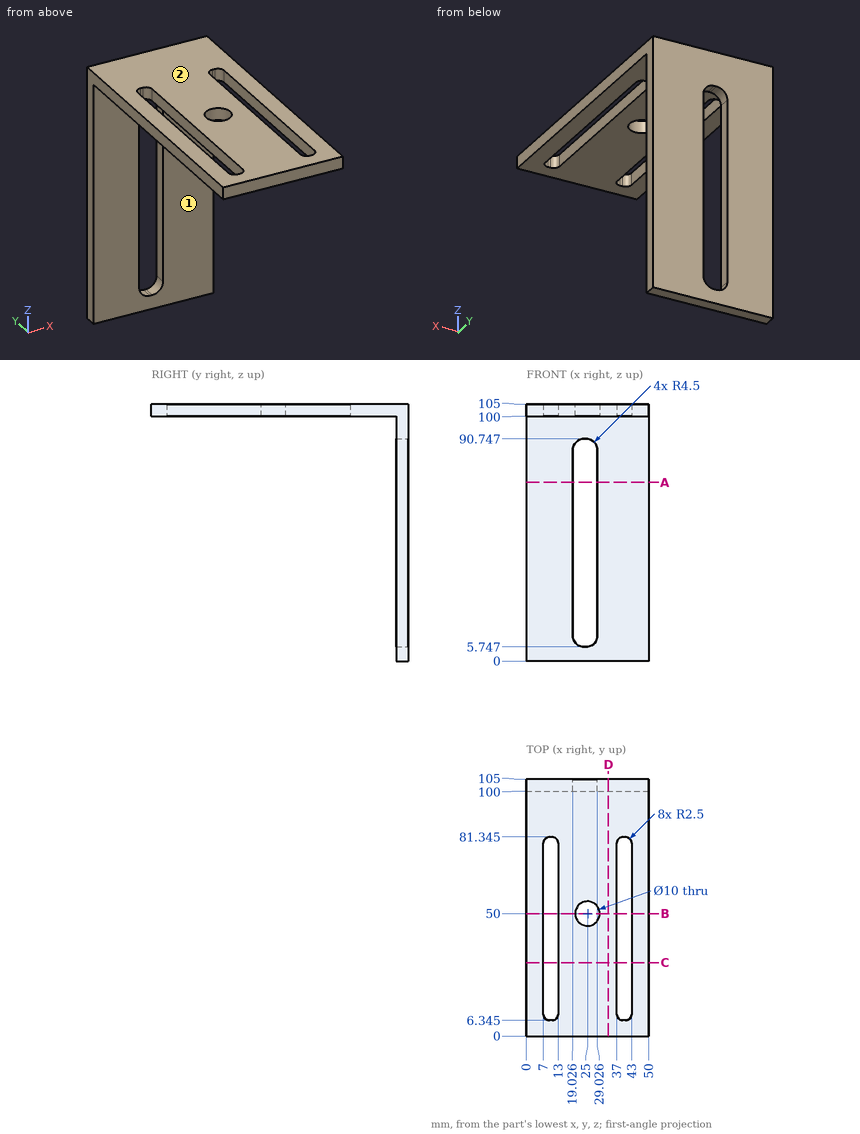
Design review of the part shown in the three views and the two pictorial views. Dimensions are in mm from the part's minimum x, y and z. A direction names the side the tool comes from. Round coordinates to 2 decimals unless told otherwise and drop trailing zeros. Order: outer loops, then holes, each group sorted by start corner. A loop starts at its lowest first (then second) coordinate and runs counter-clockwise, first axis right, second up.
(1) Take a section at A-A, the plane z = 73. State the section outline as (x, y) points, plus the area to 3 significant figures.
Working result:
outline: (0, 100) - (19.03, 100) - (19.03, 105) - (0, 105) - close; (29.03, 100) - (50, 100) - (50, 105) - (29.03, 105) - close
area: 200 mm2
(2) For P1, Ø5, axis at x = 9, z = 89.5, coming from the -Y side; P2, Ø12, axis at x = 40.5, y = 36.5, coming from the -Z side; P3, Ø9, axis at x = 25, y = 50, coming from the -Z side, all flat-tipped, find the tip position at first contact; note any pin that passes through.
Working result:
P1: stops at y = 100
P2: stops at z = 100
P3: passes through
(3) Wall thickness on L1, parallel to Y at x = 25, z = 102; L2, parallel to Z at x = 45, y = 27.5: over which ranges is each line inside the solid? List them lowest first.
Working result:
L1: y = 0 to 45, 55 to 105
L2: z = 100 to 105
(4) Take a section at C-C, the plane y = 30. State the section outline as (x, z) points, plus the area to 3 significant figures.
Working result:
outline: (0, 100) - (7, 100) - (7, 105) - (0, 105) - close; (13, 100) - (37, 100) - (37, 105) - (13, 105) - close; (43, 100) - (50, 100) - (50, 105) - (43, 105) - close
area: 190 mm2
(5) Tool access review of the marked faces 1 and 2: name each direction out of +Z, -Z, +X, -X, +Y, -Y from which nothing blocks a thin tool from reaching the whole face with its end or side.
Working result:
face 1: -Z, +X, -X, -Y
face 2: +Z, +X, -X, +Y, -Y
(6) Take a section at B-B, the plane y = 50. State the section outline as (x, z) points.
Working result:
outline: (0, 100) - (7, 100) - (7, 105) - (0, 105) - close; (13, 100) - (20, 100) - (20, 105) - (13, 105) - close; (30, 100) - (37, 100) - (37, 105) - (30, 105) - close; (43, 100) - (50, 100) - (50, 105) - (43, 105) - close
(7) Take a section at D-D, the plane x = 33.5. State the section outline as (y, z) points.
Working result:
outline: (0, 100) - (100, 100) - (100, 0) - (105, 0) - (105, 105) - (0, 105) - close
